Check sheet for the modelled part. Datum: model origin and axes. Units: mm. A direction names the side the tool comes from. Give positions to 0.01 mm unless a question says otherwise; leave off trailing zeros. Write each loop counter-clockwise with the first axis right and the second up, starting at its lowest first coordinate (ties: lowest second). Pieces come first, ordered by that corner, then holes. Notation, with made-up numbers: M -30.5,79.25 L -7.5,79.25 A27 ccw -7.5,106.25 Z; hole C 4,36.25 d1. An arc over 180 degrees is marked long. Write each question's results on one line, items separated by ' | '. Start each with the question number.
from build123d import *

# Parameters (mm, degrees)
BOSS_EXTRUDE1_DEPTH = 716
SKETCH2_R           = 4.5
CUT_EXTRUDE1_DEPTH  = 716


with BuildPart() as part:
    # Sketch1 → Boss-Extrude1 (new body)
    with BuildSketch(Plane.XY):
        with BuildLine():
            Line((0, 0), (-55, 0))
            ThreePointArc((-55, 0), (-61.363961031, -2.636038969), (-64, -9))
            Line((-64, -9), (-64, -111))
            ThreePointArc((-64, -111), (-61.363961031, -117.363961031), (-55, -120))
            Line((-55, -120), (287, -120))
            ThreePointArc((287, -120), (293.363961031, -117.363961031), (296, -111))
            Line((296, -111), (296, -4))
            Line((296, -4), (292, -4))
            Line((292, -4), (292, -111))
            ThreePointArc((292, -111), (290.535533906, -114.535533906), (287, -116))
            Line((287, -116), (-55, -116))
            ThreePointArc((-55, -116), (-58.535533906, -114.535533906), (-60, -111))
            Line((-60, -111), (-60, -9))
            ThreePointArc((-60, -9), (-58.535533906, -5.464466094), (-55, -4))
            Line((-55, -4), (0, -4))
            Line((0, -4), (0, 0))
        make_face()
    extrude(amount=BOSS_EXTRUDE1_DEPTH)

    # Sketch2 → Cut-Extrude1 (cut)
    with BuildSketch(Plane.ZY.offset(64)):
        with Locations(Location((58, -60, 0), (0, 0, 270))):
            Circle(SKETCH2_R)
        with Locations(Location((258, -60, 0), (0, 0, 270))):
            Circle(SKETCH2_R)
        with Locations(Location((458, -60, 0), (0, 0, 270))):
            Circle(SKETCH2_R)
        with Locations(Location((658, -60, 0), (0, 0, 270))):
            Circle(SKETCH2_R)
    extrude(amount=-CUT_EXTRUDE1_DEPTH, mode=Mode.SUBTRACT)


solid = part.part
Q1. Tool access check on faces 4 (the face through (88, -117, 716)), 5 (the face through (292, -57, 353)), 6 (the face through (-28, -4, 353)). Record the directions out of +Z, -Z, +X, -X, +Y, -Y that give a thin tool (end or side, any length) a straight path to the whole face; none if there is none.
Q2. Section check A-A on y = -33.5. Record the boundary of the cut face in (x, z).
Q3. Scan lines: L1, parallel to Z at x = 293, y = -60; L2, parallel to X at y = -76, z = 627.5; L3, parallel to Y at x = 294.15, z = 258. Record each from-to range of solid material in increasing order.
Q4. Section check C-C on x = 82. Record the boundary of the cut face in (y, z).
Q5. Release check for a two-part mould opening along Y. For faces 1 (the face through (-60, -61, 353)), 2 (the face through (114, -120, 353)), 3 (the face through (88, -117, 0)) record: pulls with the +Y half, pulls with the -Y half, needs draft (parallel to the pull), parting line crosses it, or undercut.
Q6. Section check B-B on z = 214. Record the boundary of the cut face in (x, y).
Q7. Depth check by flat-ended pin: pin 1 Ø1.5 at (x, z) = (192.5, 624.5) entering from +Y; pin 2 Ø2 at (x, z) = (294, 321.5) entering from +Y; pin 3 Ø1.2 at (y, z) = (-3, 418) entering from +X. Enter the tip coordinate at first touch or a pass-through.
Check result:
1) face 4: +Z, +X, -X, +Y, -Y | face 5: +Z, -Z, +Y | face 6: +Z, -Z
2) outline: M -64,0 L -60,0 L -60,716 L -64,716 Z; M 292,0 L 296,0 L 296,716 L 292,716 Z
3) L1: 0 to 53.5, 62.5 to 253.5, 262.5 to 453.5, 462.5 to 653.5, 662.5 to 716 | L2: -64 to -60, 292 to 296 | L3: -116.47 to -64.5, -55.5 to -4
4) outline: M -120,0 L -116,0 L -116,716 L -120,716 Z
5) face 1: undercut | face 2: pulls with the -Y half | face 3: needs draft
6) outline: M -64,-111 A9 ccw -55,-120 L 287,-120 A9 ccw 296,-111 L 296,-4 L 292,-4 L 292,-111 A5 cw 287,-116 L -55,-116 A5 cw -60,-111 L -60,-9 A5 cw -55,-4 L 0,-4 L 0,0 L -55,0 A9 ccw -64,-9 Z
7) pin 1: y = -116 | pin 2: y = -4 | pin 3: x = 0
